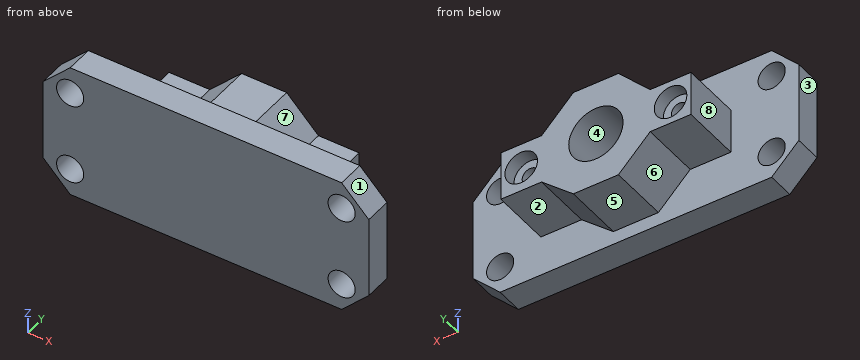
```python
from build123d import *

# Parameters (mm, degrees)
BASE_PLATE_SKETCH_W        = 120
BASE_PLATE_SKETCH_H        = 10
BASE_PLATE_DEPTH           = 50
MOUNTING_HOLES_SKETCH_R    = 5
MOUNTING_HOLES_4X_10_DEPTH = 131.384048104
CENTER_SUPPORT_DEPTH       = 22
CENTER_BORE_SKETCH_R       = 10
CENTER_BORE_20_DEPTH       = 22
SUPPORT_HOLES_SKETCH_R     = 3
SUPPORT_HOLES_2X_6_DEPTH   = 30
COUNTERBORE_SKETCH_R       = 6
COUNTERBORES_2X_12X5_DEPTH = 5
CORNER_CHAMFERS_10MM_SIZE  = 10


with BuildPart() as part:
    # Base Plate Sketch → Base Plate (new body)
    with BuildSketch(Plane.XY):
        with Locations((60, 5)):
            Rectangle(BASE_PLATE_SKETCH_W, BASE_PLATE_SKETCH_H)
    extrude(amount=BASE_PLATE_DEPTH)

    # Mounting Holes Sketch → Mounting Holes 4xØ10 (cut, through all)
    with BuildSketch(Plane(origin=(0, 10, 0), x_dir=(1, 0, 0), z_dir=(0, 1, 0))):
        with Locations(Location((10, -10, 0), (0, 0, 270))):
            Circle(MOUNTING_HOLES_SKETCH_R)
        with Locations(Location((10, -40, 0), (0, 0, 270))):
            Circle(MOUNTING_HOLES_SKETCH_R)
        with Locations(Location((110, -10, 0), (0, 0, 270))):
            Circle(MOUNTING_HOLES_SKETCH_R)
        with Locations(Location((110, -40, 0), (0, 0, 270))):
            Circle(MOUNTING_HOLES_SKETCH_R)
    extrude(amount=-MOUNTING_HOLES_4X_10_DEPTH, mode=Mode.SUBTRACT)

    # Center Support Sketch → Center Support (add)
    with BuildSketch(Plane(origin=(0, 10, 0), x_dir=(1, 0, 0), z_dir=(0, 1, 0))):
        Polygon((25, -16.7), (40, -16.7), (51.7, -5), (68.3, -5), (80, -15), (95, -15), (95, -33.3), (80, -33.3), (68.3, -45), (51.7, -45), (40, -33.3), (25, -33.3), align=None)
    extrude(amount=CENTER_SUPPORT_DEPTH)

    # Center Bore Sketch → Center Bore Ø20 (cut)
    with BuildSketch(Plane(origin=(0, 32, 0), x_dir=(1, 0, 0), z_dir=(0, 1, 0))):
        with Locations(Location((60, -25, 0), (0, 0, 270))):
            Circle(CENTER_BORE_SKETCH_R)
    extrude(amount=-CENTER_BORE_20_DEPTH, mode=Mode.SUBTRACT)

    # Support Holes Sketch → Support Holes 2xØ6 (cut)
    with BuildSketch(Plane(origin=(0, 32, 0), x_dir=(1, 0, 0), z_dir=(0, 1, 0))):
        with Locations(Location((32.5, -25, 0), (0, 0, 270))):
            Circle(SUPPORT_HOLES_SKETCH_R)
        with Locations(Location((87.5, -24.15, 0), (0, 0, 270))):
            Circle(SUPPORT_HOLES_SKETCH_R)
    extrude(amount=-SUPPORT_HOLES_2X_6_DEPTH, mode=Mode.SUBTRACT)

    # Counterbore Sketch → Counterbores 2xØ12x5 (cut)
    with BuildSketch(Plane(origin=(0, 32, 0), x_dir=(1, 0, 0), z_dir=(0, 1, 0))):
        with Locations(Location((32.5, -25, 0), (0, 0, 270))):
            Circle(COUNTERBORE_SKETCH_R)
        with Locations(Location((87.5, -24.15, 0), (0, 0, 270))):
            Circle(COUNTERBORE_SKETCH_R)
    extrude(amount=-COUNTERBORES_2X_12X5_DEPTH, mode=Mode.SUBTRACT)

    # Corner Chamfers 10mm
    corner_chamfers_10mm_edges = [part.edges().sort_by_distance(p)[0] for p in [
        (120, 5, 50),
        (0, 5, 50),
        (120, 5, 0),
        (0, 5, 0),
    ]]
    chamfer(corner_chamfers_10mm_edges, length=CORNER_CHAMFERS_10MM_SIZE)


solid = part.part
```
Check sheet for the modelled part. Datum: model origin and axes. Units: mm. Face numbers are marked on the shaded views. A direction names the side the tool comes from. Round coordinates to 2 decimals unless told otherwise and drop trailing zeros. Order: outer loops, then holes, each group sorted by start corner. A loop starts at its lowest first (then second) coordinate and runs counter-clockwise, first axis right, second up. Notation, with made-up numbers: (19, -37.5) -> (61, -37.5) arc R21 ccw to (61, -29.5) -> close; hole circle Ø11 at (79, 60). An arc over 180 degrees is marked (long way). One line per item, written item: value. Start each with the question number.
Q1. Mould release check, pull along X, two halves, no side actions. Record for the marked faces 1, 2, 3 and 4: pulls with the +X half, pulls with the -X half, needs draft (parallel to the pull), parting line crosses it, or undercut.
Q2. Gauge pin test, flat ends, axial feed: pin 1 Ø16.5 at (x, y) = (86.5, 17) entering from +Z; pin 2 Ø13.5 at (x, y) = (62, 21) entering from +Z; pin 3 Ø16.5 at (x, y) = (85, 26) entering from -Z; pin 4 Ø3.5 at (x, z) = (87.5, 24.15) entering from +Y. Record the tip position at first contact, or that the pin passes through.
Q3. Cross-section at B-B (y = 4). Record the boundary of the cut face in (x, z), and give its area (3 significant figures).
Q4. Cross-section at A-A (z = 7). Record the boundary of the cut face in (x, y).
Q5. Set-up check for the marked faces 5, 6, 7 and 8: record each of +Z, -Z, +X, -X, +Y, -Y from which the full face is reachable in a straight line by a thin tool's end or side.
Q6. Cross-section at C-C (y = 17). Record the boundary of the cut face in (x, z), and give its area (3 significant figures).
Q7. Thickness scan on line 1 (X direction, y = 7, z = 10); line 2 (X direction, y = 18, z = 24); line 3 (Y direction, x = 82, z = 25.5). Record the ranges inside material, lowest first.
Q8. Cross-section at D-D (x = 87.5). Record the boundary of the cut face in (y, z), and give its area (3 significant figures).
Completed:
1. face 1: pulls with the +X half
1. face 2: needs draft
1. face 3: pulls with the -X half
1. face 4: undercut
2. pin 1: stops at z = 50
2. pin 2: stops at z = 45
2. pin 3: stops at z = 12.22
2. pin 4: stops at y = 2
3. outline: (0, 10) -> (10, 0) -> (110, 0) -> (120, 10) -> (120, 40) -> (110, 50) -> (10, 50) -> (0, 40) -> close; hole circle Ø10 at (10, 10); hole circle Ø10 at (10, 40); hole circle Ø6 at (32.5, 25); hole circle Ø6 at (87.5, 24.15); hole circle Ø10 at (110, 10); hole circle Ø10 at (110, 40)
3. area: 5,430 mm²
4. outline: (3, 0) -> (6, 0) -> (6, 10) -> (3, 10) -> close; (14, 0) -> (106, 0) -> (106, 10) -> (70.64, 10) -> (70.64, 32) -> (49.7, 32) -> (49.7, 10) -> (14, 10) -> close; (114, 0) -> (117, 0) -> (117, 10) -> (114, 10) -> close
5. face 5: -Z, +X, -X, +Y
5. face 6: -Z, -X, +Y
5. face 7: +Z, +X, +Y
5. face 8: +Z, -Z, -X, +Y
6. outline: (25, 16.7) -> (40, 16.7) -> (51.7, 5) -> (68.3, 5) -> (80, 15) -> (95, 15) -> (95, 33.3) -> (80, 33.3) -> (68.3, 45) -> (51.7, 45) -> (40, 33.3) -> (25, 33.3) -> close; hole circle Ø6 at (32.5, 25); hole circle Ø20 at (60, 25); hole circle Ø6 at (87.5, 24.15)
6. area: 1,490 mm²
7. line 1: x = 0 to 5, 15 to 105, 115 to 120
7. line 2: x = 25 to 29.67, 35.33 to 50.05, 69.95 to 84.5, 90.5 to 95
7. line 3: y = 0 to 27
8. outline: (0, 0) -> (10, 0) -> (10, 15) -> (32, 15) -> (32, 18.15) -> (27, 18.15) -> (27, 21.15) -> (2, 21.15) -> (2, 27.15) -> (27, 27.15) -> (27, 30.15) -> (32, 30.15) -> (32, 33.3) -> (10, 33.3) -> (10, 50) -> (0, 50) -> close
8. area: 693 mm²
